```python
from build123d import *

# Parameters (mm, degrees)
SKETCH_1_R      = 4
SKETCH_1_R_2    = 2.15
EXTRUDE_1_DEPTH = 0.5
SKETCH_2_W      = 21
SKETCH_2_H      = 6
EXTRUDE_2_DEPTH = 0.5


with BuildPart() as part:
    # 草图1 → 凸台-拉伸1 (new, symmetric)
    with BuildSketch(Plane.XY):
        Circle(SKETCH_1_R)
        Circle(SKETCH_1_R_2, mode=Mode.SUBTRACT)
    extrude(amount=EXTRUDE_1_DEPTH, both=True)

    # 草图2 → 凸台-拉伸2 (add, symmetric)
    with BuildSketch(Plane.XY):
        with Locations((13.5, 0)):
            Rectangle(SKETCH_2_W, SKETCH_2_H)
    extrude(amount=EXTRUDE_2_DEPTH, both=True)


solid = part.part
```
The model under review builds one solid part; all positions refer to its coordinate system, in mm. A direction names the side the tool comes from. Round coordinates to 2 decimals unless told otherwise and drop trailing zeros. Loops run counter-clockwise (first coordinate to the right, second up) from the corner with the lowest first, then second, coordinate; pieces in that order, holes last.
Item 1: For line 1 (Y direction, x = 0, z = 0.05); line 2 (X direction, y = 1, z = 0.4); line 3 (Y direction, x = 19, z = 0.45), list the stretches that pass through material, from the lowest coordinate up.
Determined:
line 1: y = -4 to -2.15, 2.15 to 4
line 2: x = -3.87 to -1.9, 1.9 to 24
line 3: y = -3 to 3
Item 2: Take a section at C-C (x = 0). Write out the cut boundary in (y, z), then the cut area to 3 significant figures.
Determined:
outline: (-4, -0.5) - (-2.15, -0.5) - (-2.15, 0.5) - (-4, 0.5) - close; (2.15, -0.5) - (4, -0.5) - (4, 0.5) - (2.15, 0.5) - close
area: 3.70 mm2
Item 3: Take a section at D-D (x = 9.75). Write out the cut boundary in (y, z).
Determined:
outline: (-3, -0.5) - (3, -0.5) - (3, 0.5) - (-3, 0.5) - close
Item 4: Take a section at A-A (y = 0). Write out the cut boundary in (x, z), then the cut area to 3 significant figures.
Determined:
outline: (-4, -0.5) - (-2.15, -0.5) - (-2.15, 0.5) - (-4, 0.5) - close; (2.15, -0.5) - (24, -0.5) - (24, 0.5) - (2.15, 0.5) - close
area: 23.7 mm2
Item 5: Clearance check with flat-ended pins moving along their axes: pin 1 Ø0.5 at (x, z) = (12.5, 0) entering from -Y; pin 2 Ø0.5 at (x, z) = (17, 0) entering from +Y. State where each tip first meets the part, or that it passes through.
Determined:
pin 1: stops at y = -3
pin 2: stops at y = 3
Item 6: For faces 1 (the face through (10, 0, -0.5)), 2 (the face through (13, -3, 0)), list the 3-axis set-ups (+Z, -Z, +X, -X, +Y, -Y) from which the entire face can be reached by the end or side of a thin tool; tool diameter is ignored.
Determined:
face 1: -Z, +X, -X, +Y, -Y
face 2: +Z, -Z, +X, -Y
Item 7: Take a section at B-B (z = 0.1). Write out the cut boundary in (x, y), then the cut area to 3 significant figures.
Determined:
outline: (3, -3) - (24, -3) - (24, 3) - (3, 3) - (3, 2.65) arc R4 ccw (long way) to (3, -2.65) - close; hole circle Ø4.3 at (0, 0)
area: 158 mm2
Item 8: Mouldability with a two-part tool opening along X and no side actions: class faces 3 (the face through (13, 3, 0)), 4 (the face through (24, 0, 0)), 5 (the face through (-2.15, 0.09, -0.01)) as released by +X, released by -X, zero draft, split by the parting line, or undercut.
Determined:
face 3: zero draft
face 4: released by +X
face 5: undercut
